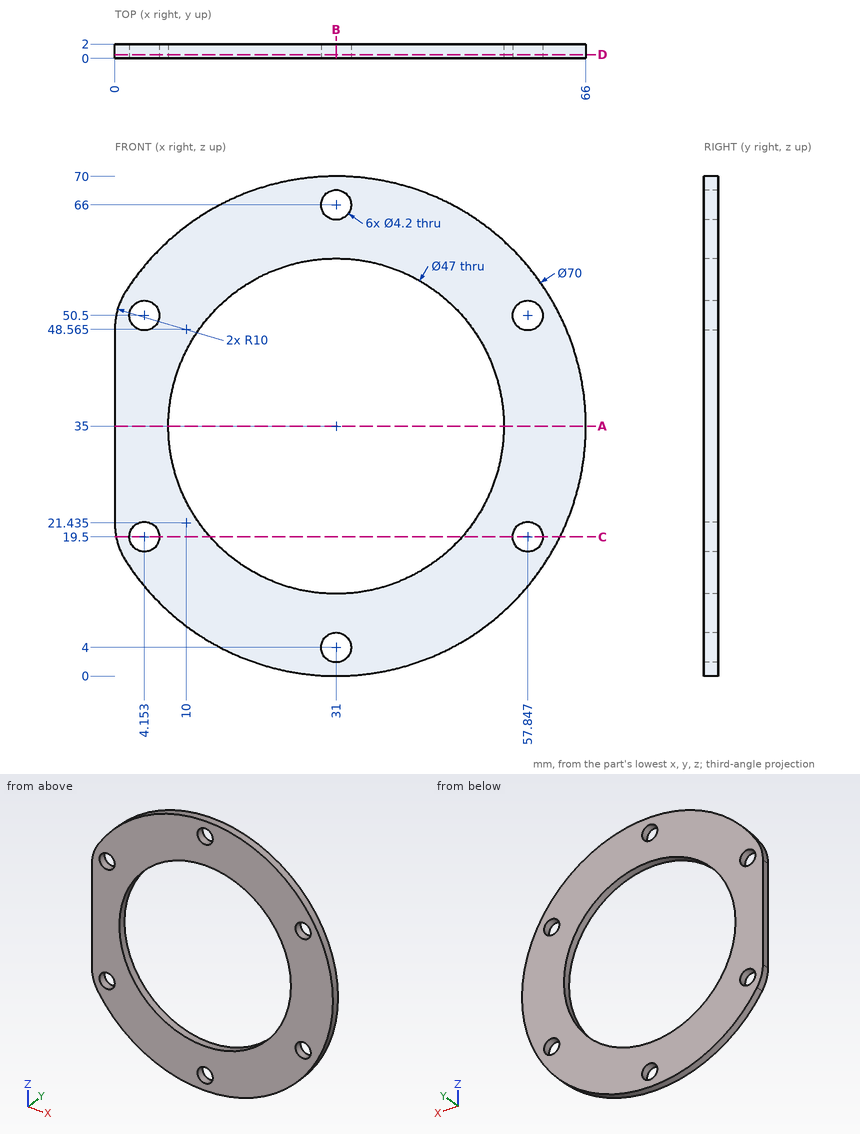
Could you check a few things on this drawing? It's one solid part, dimensions in mm from its lowest x, y, z. Round coordinates to 2 decimals unless told otherwise and drop trailing zeros. Write each loop counter-clockwise with the first axis right and the second up, starting at its lowest first coordinate (ties: lowest second). Pieces come first, ordered by that corner, then holes. Notation, with made-up numbers: (-29.5, 80) -> (3.5, 80) arc R20 ccw to (3.5, 116) -> close; hole circle Ø6 at (36.5, 45). An arc over 180 degrees is marked (long way). Use a Markdown table: item, result.
1. If we section it at A-A (z = 35): List the corners of the cut face in (x, y) for me.
Answer key:
| item | result |
|---|---|
| outline | (0, 0) -> (7.5, 0) -> (7.5, 2) -> (0, 2) -> close; (54.5, 0) -> (66, 0) -> (66, 2) -> (54.5, 2) -> close |
2. Please list where these lines run through material, in increasing order: probe 1 along Z at (x, y) = (5, 1.7); probe 2 along Z at (x, y) = (3, 0.65) (1 decimal); probe 3 along X at (y, z) = (1.8, 20.5) (1 decimal).
Answer key:
| item | result |
|---|---|
| probe 1 | z = 11.57 to 17.58, 21.42 to 48.58, 52.42 to 58.43 |
| probe 2 | z = 14 to 17.7, 21.3 to 48.7, 52.3 to 56 |
| probe 3 | x = 0 to 2.3, 6 to 12.5, 49.5 to 56, 59.7 to 62.9 |
3. If we section it at D-D (y = 0.5): List the corners of the cut face in (x, z) for me (1 decimal), then the cut area to 3 significant figures.
Answer key:
| item | result |
|---|---|
| outline | (0, 21.4) arc R10 ccw to (1.6, 16) arc R35 ccw (long way) to (1.6, 54) arc R10 ccw to (0, 48.6) -> close; hole circle Ø4.2 at (4.2, 19.5); hole circle Ø4.2 at (4.2, 50.5); hole circle Ø47 at (31, 35); hole circle Ø4.2 at (31, 4); hole circle Ø4.2 at (31, 66); hole circle Ø4.2 at (57.8, 19.5); hole circle Ø4.2 at (57.8, 50.5) |
| area | 1,940 mm^2 |
4. If we section it at C-C (z = 19.5): List the corners of the cut face in (x, y) for me.
Answer key:
| item | result |
|---|---|
| outline | (0.19, 0) -> (2.05, 0) -> (2.05, 2) -> (0.19, 2) -> close; (6.25, 0) -> (13.34, 0) -> (13.34, 2) -> (6.25, 2) -> close; (48.66, 0) -> (55.75, 0) -> (55.75, 2) -> (48.66, 2) -> close; (59.95, 0) -> (62.38, 0) -> (62.38, 2) -> (59.95, 2) -> close |
5. If we section it at B-B (x = 31): List the corners of the cut face in (y, z) for me.
Answer key:
| item | result |
|---|---|
| outline | (0, 0) -> (2, 0) -> (2, 1.9) -> (0, 1.9) -> close; (0, 6.1) -> (2, 6.1) -> (2, 11.5) -> (0, 11.5) -> close; (0, 58.5) -> (2, 58.5) -> (2, 63.9) -> (0, 63.9) -> close; (0, 68.1) -> (2, 68.1) -> (2, 70) -> (0, 70) -> close |
